Geometry: final body of the model. Coordinates: model frame, mm. Face numbers are marked on the shaded views. A direction names the side the tool comes from. Give positions to 0.01 mm unless a question says otherwise; leave off trailing zeros. Loops run counter-clockwise (first coordinate to the right, second up) from the corner with the lowest first, then second, coordinate; pieces in that order, holes last. Notation, with made-up numbers: (-29, 88.25) -> (2, 88.25) arc R31 ccw to (2, 127.25) -> close; hole circle Ø4 at (-27.5, 30). An arc over 180 degrees is marked (long way). Answer in a Markdown table with one row per item. Add a question column.
1) Section query B-B (y = 80). Give the number of separate pieces and of enclosed holes in the cut face, plus the area to 3 significant figures.
2) Line query: line 1 (X direction, y = 50, z = -23.2); line 2 (X direction, y = 28.5, z = -11); line 3 (Z direction, x = 94, y = 70.5). Output: solid intervals per line, ascending. Write a range as from..to.
3) Section query A-A (x = 65). Return the cut outline in (y, z).
4) Section query D-D (z = 0). Return the cut outline in (x, y).
5) First-contact query: P1, Ø3, axis at y = 66, z = -21.5, coming from the +X side; P2, Ø4, axis at x = 98, z = 25.5, coming from the -Y side; P3, Ø24, axis at y = 57.5, z = -0.5, coming from the +X side. Flat tips, straight axial feed; report the tip coordinate or a pass-through.
6) Section query C-C (x = 13). Return the cut outline in (y, z).
7) Draft query along X for the marked faces 1, 2 and 3. Return one class per face: +X half, -X half, draft (parallel to the pull), parting line (faces both ways), or undercut.
8) Access query for the marked faces 4, 5, 6, 7 and 8. Directions: +Z, -Z, +X, -X, +Y, -Y. A direction counts if a zero-diameter tool reaches every point of the face in a straight line with its end or side. Return the directions, or none.
```python
from build123d import *

# Parameters (mm, degrees)
BASE_BLOCK_100_DEPTH          = 50
BOTTOM_ARCH_CUT_DEPTH         = 145.913767462
LEFT_UPRIGHT_SKETCH_W         = 50
LEFT_UPRIGHT_SKETCH_H         = 1.583123952
LEFT_UPRIGHT_60_DEPTH         = 60
RIGHT_UPRIGHT_60_DEPTH        = 60
LEFT_UPRIGHT_RECESS_SKETCH_R  = 15
LEFT_UPRIGHT_RECESS_5_DEPTH   = 5
RIGHT_START                   = -5
RIGHT_UPRIGHT_RECESS_SKETCH_R = 15
RIGHT_UPRIGHT_RECESS_5_DEPTH  = 5
SIDE_WEB_20_DEPTH             = 20
WEB_SADDLE_SKETCH_R           = 30
WEB_SADDLE_CUT_DEPTH          = 176.695759767
CENTRE_RIB_SKETCH_W           = 130
CENTRE_RIB_SKETCH_H           = 26
CENTRE_RIB_10_DEPTH           = 10
RIB_NOTCH_A_DEPTH             = 176.695759767
RIB_NOTCH_B_DEPTH             = 176.695759767
CROSS_HOLE_SKETCH_R           = 30
CROSS_HOLE_30_DEPTH           = 172.464281995


with BuildPart() as part:
    # Base Profile Sketch → Base Block 100 (new, symmetric)
    with BuildSketch(Plane.XY):
        Polygon((0, 40), (0, 0), (130, 0), (130, 40), (90, 40), (90, 25), (65, 25), (40, 25), (40, 40), align=None)
    base_block_100 = extrude(amount=BASE_BLOCK_100_DEPTH, both=True)

    # Bottom Arch Sketch → Bottom Arch Cut (cut, through all)
    with BuildSketch(Plane(origin=(130, 0, 0), x_dir=(0, 0, -1), z_dir=(1, 0, 0))):
        with BuildLine():
            Line((-30, 0), (30, 0))
            ThreePointArc((30, 0), (0, 30), (-30, 0))
        make_face()
        with BuildLine():
            ThreePointArc((-30, 0), (0, -30), (30, 0))
            Line((30, 0), (-30, 0))
        make_face()
    extrude(amount=-BOTTOM_ARCH_CUT_DEPTH, mode=Mode.SUBTRACT)

    # Left Upright Sketch → Left Upright 60 (add)
    with BuildSketch(Plane(origin=(0, 25, 0), x_dir=(1, 0, 0), z_dir=(0, 1, 0))):
        with Locations((65, -15.791561976)):
            Rectangle(LEFT_UPRIGHT_SKETCH_W, LEFT_UPRIGHT_SKETCH_H)
        Polygon((40, -25), (65, -25), (90, -25), (90, -16.583123952), (40, -16.583123952), align=None)
    extrude(amount=LEFT_UPRIGHT_60_DEPTH)

    # Right Upright Sketch → Right Upright 60 (add)
    with BuildSketch(Plane(origin=(0, 25, 0), x_dir=(1, 0, 0), z_dir=(0, 1, 0))):
        Polygon((90, 25), (65, 25), (40, 25), (40, 15), (90, 15), align=None)
    extrude(amount=RIGHT_UPRIGHT_60_DEPTH)

    # Left Upright Recess Sketch → Left Upright Recess 5 (cut)
    with BuildSketch(Plane.XY.offset(25)):
        with Locations((65, 50)):
            Circle(LEFT_UPRIGHT_RECESS_SKETCH_R)
    extrude(amount=-LEFT_UPRIGHT_RECESS_5_DEPTH, mode=Mode.SUBTRACT)

    # Right Upright Recess Sketch → Right Upright Recess 5 (cut)
    with BuildSketch(Plane(origin=(0, 0, -25), x_dir=(-1, 0, 0), z_dir=(0, 0, -1)).offset(RIGHT_START)):
        with Locations(Location((-65, 50, 0), (0, 0, 180))):
            Circle(RIGHT_UPRIGHT_RECESS_SKETCH_R)
    extrude(amount=RIGHT_UPRIGHT_RECESS_5_DEPTH, mode=Mode.SUBTRACT)

    # Side Web Sketch → Side Web 20 (add)
    with BuildSketch(Plane.XY.offset(13)):
        Polygon((40, 40), (40, 100), (25, 100), (0, 40), align=None)
        Polygon((90, 40), (90, 100), (105, 100), (130, 40), align=None)
    side_web_20 = extrude(amount=SIDE_WEB_20_DEPTH)

    # Web Saddle Sketch → Web Saddle Cut (cut, symmetric)
    with BuildSketch(Plane.XY.offset(13)):
        with Locations((65, 100)):
            Circle(WEB_SADDLE_SKETCH_R)
    web_saddle_cut = extrude(amount=WEB_SADDLE_CUT_DEPTH, both=True, mode=Mode.SUBTRACT)

    # Side Web and Saddle Mirror: Base Block 100, Side Web 20, Web Saddle Cut across plane
    add(base_block_100.mirror(Plane.XY))
    add(side_web_20.mirror(Plane.XY))
    add(web_saddle_cut.mirror(Plane.XY), mode=Mode.SUBTRACT)

    # Centre Rib Sketch → Centre Rib 10 (add)
    with BuildSketch(Plane(origin=(0, 40, 0), x_dir=(1, 0, 0), z_dir=(0, 1, 0))):
        with Locations((65, 0)):
            Rectangle(CENTRE_RIB_SKETCH_W, CENTRE_RIB_SKETCH_H)
    extrude(amount=CENTRE_RIB_10_DEPTH)

    # Rib Notch A Sketch → Rib Notch A (cut, through all)
    with BuildSketch(Plane.XY.offset(13)):
        Polygon((4.166666667, 50), (0, 50), (0, 40), align=None)
    extrude(amount=-RIB_NOTCH_A_DEPTH, mode=Mode.SUBTRACT)

    # Rib Notch B Sketch → Rib Notch B (cut, through all)
    with BuildSketch(Plane.XY.offset(13)):
        Polygon((125.833333333, 50), (130, 40), (130, 50), align=None)
    extrude(amount=-RIB_NOTCH_B_DEPTH, mode=Mode.SUBTRACT)

    # Cross Hole Sketch → Cross Hole Ø30 (cut, through all)
    with BuildSketch(Plane(origin=(130, 0, 0), x_dir=(0, 0, -1), z_dir=(1, 0, 0))):
        Circle(CROSS_HOLE_SKETCH_R)
    extrude(amount=-CROSS_HOLE_30_DEPTH, mode=Mode.SUBTRACT)


solid = part.part
```
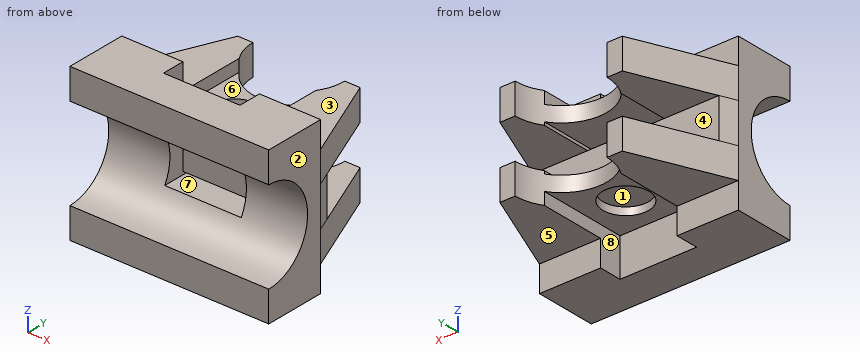
Evaluation:
| question | item | result |
|---|---|---|
| 1 | separate pieces | 4 |
| 1 | enclosed holes | 0 |
| 1 | area | 1,970 mm² |
| 2 | line 1 | 4.17..50, 80..125.83 |
| 2 | line 2 | 0..40, 90..130 |
| 2 | line 3 | -33..-13, 13..33 |
| 3 | outline | (0, -50) -> (25, -50) -> (25, -25) -> (35, -25) -> (35, -20) -> (65, -20) -> (65, -25) -> (70, -25) -> (70, -15) -> (25.98, -15) arc R30 cw to (0, -30) -> close; (0, 30) arc R30 cw to (25.98, 15) -> (70, 15) -> (70, 25) -> (65, 25) -> (65, 20) -> (35, 20) -> (35, 25) -> (25, 25) -> (25, 50) -> (0, 50) -> close; (40, -13) -> (50, -13) -> (50, 13) -> (40, 13) -> close |
| 4 | outline | (0, 30) -> (40, 30) -> (40, 40) -> (90, 40) -> (90, 30) -> (130, 30) -> (130, 40) -> (125.83, 50) -> (4.17, 50) -> (0, 40) -> close |
| 5 | P1 | x = 119.79 |
| 5 | P2 | y = 11.99 |
| 5 | P3 | x = 127.71 |
| 6 | outline | (0, -50) -> (40, -50) -> (40, -33) -> (71.2, -33) -> (71.2, -13) -> (50, -13) -> (50, 13) -> (71.2, 13) -> (71.2, 33) -> (40, 33) -> (40, 50) -> (0, 50) -> (0, 30) arc R30 cw to (0, -30) -> close |
| 7 | face 1 | undercut |
| 7 | face 2 | +X half |
| 7 | face 3 | draft |
| 8 | face 4 | +X, -X, +Y |
| 8 | face 5 | -Z, +X, -X, +Y |
| 8 | face 6 | +Z, +Y |
| 8 | face 7 | +Y, -Y |
| 8 | face 8 | -Z, +Y |
